```python
from build123d import *

# Parameters (mm, degrees)
EXTRUDE_1_DEPTH     = 4
CUT_EXTRUDE_1_REACH = 91.112
FILLET_1_R          = 5
CUT_EXTRUDE_2_REACH = 91.112
SKETCH_3_W          = 35
SKETCH_3_H          = 16
FILLET_2_R          = 2


with BuildPart() as part:
    # 草图1 → 凸台-拉伸1 (new body)
    with BuildSketch(Plane.XY):
        Polygon((0, 0), (0, -55), (70, -55), (70, -25), (20, -25), (20, 0), align=None)
    extrude(amount=EXTRUDE_1_DEPTH)

    # 草图2 → 切除-拉伸1 (cut, up to next)
    with BuildSketch(Plane.XY.offset(4), mode=Mode.PRIVATE) as cut_extrude_1_sk1:
        with BuildLine():
            Line((3, -15), (3, -5))
            ThreePointArc((3, -5), (5, -3), (7, -5))
            Line((7, -5), (7, -15))
            ThreePointArc((7, -15), (5, -17), (3, -15))
        make_face()
    cut_extrude_1_tool1 = extrude(cut_extrude_1_sk1.sketch, amount=-CUT_EXTRUDE_1_REACH, mode=Mode.PRIVATE) & part.part
    # 草图2 → 切除-拉伸1 (cut, up to next)
    with BuildSketch(Plane.XY.offset(4), mode=Mode.PRIVATE) as cut_extrude_1_sk2:
        with BuildLine():
            Line((13, -15), (13, -5))
            ThreePointArc((13, -5), (15, -3), (17, -5))
            Line((17, -5), (17, -15))
            ThreePointArc((17, -15), (15, -17), (13, -15))
        make_face()
    cut_extrude_1_tool2 = extrude(cut_extrude_1_sk2.sketch, amount=-CUT_EXTRUDE_1_REACH, mode=Mode.PRIVATE) & part.part
    add(cut_extrude_1_tool1.solids().sort_by_distance((5, -10, 4))[0], mode=Mode.SUBTRACT)
    add(cut_extrude_1_tool2.solids().sort_by_distance((15, -10, 4))[0], mode=Mode.SUBTRACT)

    # 圆角1
    fillet_1_edges = [part.edges().sort_by_distance(p)[0] for p in [
        (20, -25, 2),
    ]]
    fillet(fillet_1_edges, radius=FILLET_1_R)

    # 草图3 → 切除-拉伸2 (cut, up to next)
    with BuildSketch(Plane.XY.offset(4), mode=Mode.PRIVATE) as cut_extrude_2_sk1:
        with Locations((52.5, -40)):
            Rectangle(SKETCH_3_W, SKETCH_3_H)
    cut_extrude_2_tool1 = extrude(cut_extrude_2_sk1.sketch, amount=-CUT_EXTRUDE_2_REACH, mode=Mode.PRIVATE) & part.part
    add(cut_extrude_2_tool1.solids().sort_by_distance((52.5, -40, 4))[0], mode=Mode.SUBTRACT)

    # 圆角2
    fillet_2_edges = [part.edges().sort_by_distance(p)[0] for p in [
        (35, -48, 2),
        (35, -32, 2),
    ]]
    fillet(fillet_2_edges, radius=FILLET_2_R)


solid = part.part
```
Work out the finished part from the listing and answer in its coordinate system (mm). A direction names the side the tool comes from. Coordinates: 2 decimals unless noted, no trailing zeros. Loops run counter-clockwise (first coordinate to the right, second up) from the corner with the lowest first, then second, coordinate; pieces in that order, holes last.
1) Consider probe 1 along X at (y, z) = (-14.5, 2.15); probe 2 along Y at (x, z) = (55.5, 0.9); probe 3 along Y at (x, z) = (29, 3.05). Determine where each line is inside the solid, lowest interval first.
Results:
probe 1: x = 0 to 3, 7 to 13, 17 to 20
probe 2: y = -55 to -48, -32 to -25
probe 3: y = -55 to -25
2) Section D-D (y = -24) is taken. Give the vertices of the cut face in (x, z).
Results:
outline: (0, 0) - (22, 0) - (22, 4) - (0, 4) - close
3) Flat-ended cylindrical pins translate along their axes: pin 1 (2 mm diameter, centred on y = -7.5, z = 2.5, fed in from +X); pin 2 (1.2 mm diameter, centred on y = -39.5, z = 3, fed in from +X); pin 3 (2 mm diameter, centred on x = 36.5, z = 1.5, fed in from +Y). Find the tip coordinate at first contact, or state that the pin passes through.
Results:
pin 1: stops at x = 20
pin 2: stops at x = 35
pin 3: stops at y = -25
4) Section B-B (z = 1.3) is taken. Give the vertices of the cut face in (x, y), plus the area to 3 significant figures.
Results:
outline: (0, -55) - (70, -55) - (70, -48) - (37, -48) arc R2 cw to (35, -46) - (35, -34) arc R2 cw to (37, -32) - (70, -32) - (70, -25) - (25, -25) arc R5 cw to (20, -20) - (20, 0) - (0, 0) - close; hole (3, -15) arc R2 ccw to (7, -15) - (7, -5) arc R2 ccw to (3, -5) - close; hole (13, -15) arc R2 ccw to (17, -15) - (17, -5) arc R2 ccw to (13, -5) - close
area: 1,940 mm2
5) For a pull along Y with two mould halves and no side action, classify faces 1 (the cylindrical face through (21, -23, 2)), 2 (the cylindrical face through (15, -3, 2)), 3 (the flat face through (27, -33, 0)) as +Y half, -Y half, draft (parallel to the pull), parting line (faces both ways), or undercut.
Results:
face 1: +Y half
face 2: undercut
face 3: draft
6) Section C-C (x = 15) is taken. Give the vertices of the cut face in (y, z), plus the area to 3 significant figures.
Results:
outline: (-55, 0) - (-17, 0) - (-17, 4) - (-55, 4) - close; (-3, 0) - (0, 0) - (0, 4) - (-3, 4) - close
area: 164 mm2
7) For faces 4 (the cylindrical face through (5, -17, 2)), 5 (the flat face through (70, -52, 2)), 6 (the flat face through (27, -33, 4)), 7 (the flat face through (20, -10, 2)), 8 (the cylindrical face through (35.6, -32.57, 1.97)), determine the directions among +Z, -Z, +X, -X, +Y, -Y from which every point of the face is accessible in a straight line to the end or side of a thin tool.
Results:
face 4: +Z, -Z
face 5: +Z, -Z, +X, +Y, -Y
face 6: +Z, +X, -X, +Y, -Y
face 7: +Z, -Z, +X, +Y
face 8: +Z, -Z, +X
8) Section A-A (x = 63.5) is taken. Give the vertices of the cut face in (y, z).
Results:
outline: (-55, 0) - (-48, 0) - (-48, 4) - (-55, 4) - close; (-32, 0) - (-25, 0) - (-25, 4) - (-32, 4) - close
